```python
from build123d import *

# Parameters (mm, degrees)
EXTRUDE_1_DEPTH     = 45
FILLET_1_R          = 2
FILLET_2_R          = 7
CHAMFER_1_SIZE      = 1
CUT_EXTRUDE_1_DEPTH = 85.557672626


with BuildPart() as part:
    # 草图1 → 拉伸-薄壁1 (new body)
    with BuildSketch(Plane.XY):
        Polygon((0, 0), (0, 30), (65, 30), (65, 25), (5, 25), (5, 0), align=None)
    extrude(amount=EXTRUDE_1_DEPTH)

    # 圆角1
    fillet_1_edges = [part.edges().sort_by_distance(p)[0] for p in [
        (5, 25, 22.5),
    ]]
    fillet(fillet_1_edges, radius=FILLET_1_R)

    # 圆角2
    fillet_2_edges = [part.edges().sort_by_distance(p)[0] for p in [
        (0, 30, 22.5),
    ]]
    fillet(fillet_2_edges, radius=FILLET_2_R)

    # 倒角1
    chamfer_1_edges = [part.edges().sort_by_distance(p)[0] for p in [
        (2.5, 0, 45),
        (2.5, 0, 0),
        (65, 27.5, 0),
        (65, 27.5, 45),
    ]]
    chamfer(chamfer_1_edges, length=CHAMFER_1_SIZE)

    # 草图2 → 切除-拉伸1 (cut, through all)
    with BuildSketch(Plane(origin=(0, 30, 0), x_dir=(1, 0, 0), z_dir=(0, 1, 0))):
        with BuildLine():
            Line((22.5, -18), (57.5, -18))
            ThreePointArc((57.5, -18), (62, -22.5), (57.5, -27))
            Line((57.5, -27), (22.5, -27))
            ThreePointArc((22.5, -27), (18, -22.5), (22.5, -18))
        make_face()
    extrude(amount=-CUT_EXTRUDE_1_DEPTH, mode=Mode.SUBTRACT)


solid = part.part
```
Geometry: final body of the model. Coordinates: model frame, mm. A direction names the side the tool comes from. Coordinates: 2 decimals unless noted, no trailing zeros. Write each loop counter-clockwise with the first axis right and the second up, starting at its lowest first coordinate (ties: lowest second). Pieces come first, ordered by that corner, then holes. Notation, with made-up numbers: M -35.5,20.25 L -11.5,20.25 A25 ccw -11.5,33.25 Z; hole C 6.5,-28 d8. An arc over 180 degrees is marked long. Answer as CSV lines item,"result". Start each with the question number.
Q1. Cut plane D-D on x = 10. Return the cut outline in (y, z).
Q2. Pin query (flat end, axial travel): P1, Ø1, axis at y = 12, z = 8, coming from the +X side. Return the tip coordinate at first contact, or that it passes through.
Q3. Cut plane C-C on z = 31.5. Return the cut outline in (x, y).
Q4. Cut plane B-B on z = 22.5. Return the cut outline in (x, y), then the cut area to 3 significant figures.
Q5. Mould query, pull axis Z, two halves, no side actions, for faces 1 (the flat face through (5, 12, 22)), 2 (the flat face through (25, 25.2, 0)), 3 (the flat face through (40, 28, 18)). Classes: released by +Z, released by -Z, zero draft, split by the parting line, or undercut.
Q6. Line query: line 1 (Y direction, x = 11, z = 28.5); line 2 (X direction, y = 14.5, z = 38); line 3 (Z direction, x = 33, y = 28.75). Output: solid intervals per line, ascending. Write a range as from..to.
Q7. Reachability of faces 4 (the flat face through (36, 25, 17)), 5 (the cylindrical face through (2.1, 28, 22.8)), 6 (the cylindrical face through (18, 27.5, 22.6)) from +Z, -Z, +X, -X, +Y, -Y: full face, straight path, thin tool, end or side. Return the list, or none.
Q8. Cut plane A-A on x = 35.5. Return the cut outline in (y, z).
Findings below:
1,outline,"M 25,0 L 30,0 L 30,45 L 25,45 Z"
2,P1,"stops at x = 5"
3,outline,"M 0,0 L 5,0 L 5,23 A2 cw 7,25 L 65,25 L 65,30 L 7,30 A7 ccw 0,23 Z"
4,outline,"M 0,0 L 5,0 L 5,23 A2 cw 7,25 L 18,25 L 18,30 L 7,30 A7 ccw 0,23 Z; M 62,25 L 65,25 L 65,30 L 62,30 Z"
4,area,"220 mm2"
5,face 1,"zero draft"
5,face 2,"released by -Z"
5,face 3,"undercut"
6,line 1,"y = 25..30"
6,line 2,"x = 0..5"
6,line 3,"z = 0..18, 27..45"
7,face 4,"+Z, -Z, +X, -Y"
7,face 5,"+Z, -Z, -X, +Y"
7,face 6,"+Y, -Y"
8,outline,"M 25,0 L 30,0 L 30,18 L 25,18 Z; M 25,27 L 30,27 L 30,45 L 25,45 Z"
